```python
from build123d import *

# Parameters (mm, degrees)
SQUARE_TUBE_30_X_30_X_2_6_1_DEPTH = 200
CUT_EXTRUDE1_DEPTH                = 87
CUT_EXTRUDE2_DEPTH                = 137


with BuildPart() as part:
    # Sketch1 → Square tube 30 X 30 X 2.6(1) (new body)
    with BuildSketch(Plane.YZ):
        with BuildLine():
            Line((-21, -15), (21, -15))
            ThreePointArc((21, -15), (23.828427125, -13.828427125), (25, -11))
            Line((25, -11), (25, 11))
            ThreePointArc((25, 11), (23.828427125, 13.828427125), (21, 15))
            Line((21, 15), (-21, 15))
            ThreePointArc((-21, 15), (-23.828427125, 13.828427125), (-25, 11))
            Line((-25, 11), (-25, -11))
            ThreePointArc((-25, -11), (-23.828427125, -13.828427125), (-21, -15))
        make_face()
        with BuildLine():
            Line((-21, -12), (21, -12))
            ThreePointArc((21, -12), (21.707106781, -11.707106781), (22, -11))
            Line((22, -11), (22, 11))
            ThreePointArc((22, 11), (21.707106781, 11.707106781), (21, 12))
            Line((21, 12), (-21, 12))
            ThreePointArc((-21, 12), (-21.707106781, 11.707106781), (-22, 11))
            Line((-22, 11), (-22, -11))
            ThreePointArc((-22, -11), (-21.707106781, -11.707106781), (-21, -12))
        make_face(mode=Mode.SUBTRACT)
    extrude(amount=SQUARE_TUBE_30_X_30_X_2_6_1_DEPTH)

    # Sketch3 → Cut-Extrude1 (cut)
    with BuildSketch(Plane(origin=(0, 25, 0), x_dir=(1, 0, 0), z_dir=(0, 1, 0))):
        Polygon((188, 15), (182.710190579, -15), (200, -15), (200, 15), align=None)
    extrude(amount=-CUT_EXTRUDE1_DEPTH, mode=Mode.SUBTRACT)

    # Sketch4 → Cut-Extrude2 (cut)
    with BuildSketch(Plane(origin=(0, 25, 0), x_dir=(1, 0, 0), z_dir=(0, 1, 0))):
        Polygon((0, 15), (82.424322584, -15), (0, -15), align=None)
    extrude(amount=-CUT_EXTRUDE2_DEPTH, mode=Mode.SUBTRACT)


solid = part.part
```
Input: part model. Units: mm. Frame: model coordinates. A direction names the side the tool comes from. Coordinates: 2 decimals unless noted, no trailing zeros. Loops run counter-clockwise (first coordinate to the right, second up) from the corner with the lowest first, then second, coordinate; pieces in that order, holes last. Notation, with made-up numbers: M 31,-2 L 48,-2 A24 ccw 48,17 Z; hole C -39.75,29.25 d3. An arc over 180 degrees is marked long. Use a Markdown table: item, result. Add a question column.
1) Pin query (flat end, axial travel): P1, Ø6, axis at x = 56.5, y = -1, coming from the +Z side; P2, Ø5, axis at y = -3.5, z = -11, coming from the +X side. Return the tip coordinate at first contact, or that it passes through.
2) Section B-B, the plane x = 86.5. Return the cut outline in (y, z).
3) Section D-D, the plane x = 58. Return the cut outline in (y, z), plus the area to 3 significant figures.
4) Draft query along Y for faces 1 (the flat face through (97, 0, -12)), 2 (the flat face through (93, 0, -15)), 3 (the cylindrical face through (92.684, -23.859, -13.797)). Return one class per face: +Y half, -Y half, draft (parallel to the pull), parting line (faces both ways), or undercut.
5) Line query: L1, parallel to Y at x = 67, z = -1.75; L2, parallel to Z at x = 108, y = -14; L3, parallel to Z at x = 10, y = -16.5. Output: solid intervals per line, ascending. Write a range as from..to.
6) Set-up query: faces 4 (the flat face through (128, 0, 12)), 5 (the cylindrical face through (126.641, 23.859, 13.797)). Return all of +Z, -Z, +X, -X, +Y, -Y with unobstructed straight access to the full face (end or side cutting, diameter ignored); none if empty.
7) Section A-A, the plane y = 9. Return the cut outline in (x, z).
8) Section C-C, the plane z = 3.75. Return the cut outline in (x, y), plus the area to 3 significant figures.
Answer below:
| question | item | result |
|---|---|---|
| 1 | P1 | z = -12 |
| 1 | P2 | x = 187.74 |
| 2 | outline | M -25,-11 A4 ccw -21,-15 L 21,-15 A4 ccw 25,-11 L 25,11 A4 ccw 21,15 L -21,15 A4 ccw -25,11 Z; hole M -22,-11 A1 ccw -21,-12 L 21,-12 A1 ccw 22,-11 L 22,11 A1 ccw 21,12 L -21,12 A1 ccw -22,11 Z |
| 3 | outline | M -25,-11 A4 ccw -21,-15 L 21,-15 A4 ccw 25,-11 L 25,6.11 L 22,6.11 L 22,-11 A1 cw 21,-12 L -21,-12 A1 cw -22,-11 L -22,6.11 L -25,6.11 Z |
| 3 | area | 252 mm2 |
| 4 | face 1 | undercut |
| 4 | face 2 | draft |
| 4 | face 3 | -Y half |
| 5 | L1 | -25..-22, 22..25 |
| 5 | L2 | -15..-12, 12..15 |
| 5 | L3 | -15..-12 |
| 6 | face 4 | +X, -X |
| 6 | face 5 | +Z, +X, -X, +Y |
| 7 | outline | M 0,-15 L 188,-15 L 187.47,-12 L 8.24,-12 Z; M 74.18,12 L 183.24,12 L 182.71,15 L 82.42,15 Z |
| 8 | outline | M 51.52,-25 L 184.69,-25 L 184.69,-22 L 51.52,-22 Z; M 51.52,22 L 184.69,22 L 184.69,25 L 51.52,25 Z |
| 8 | area | 799 mm2 |
